Read the model definition and answer for the solid it produces. Units are mm, in the model's axes. Coordinates: 2 decimals unless noted, no trailing zeros. Loops run counter-clockwise (first coordinate to the right, second up) from the corner with the lowest first, then second, coordinate; pieces in that order, holes last. Notation, with made-up numbers: M -32,18.5 L -12,18.5 A16 ccw -12,27.5 Z; hole C 35.25,65 d7. An arc over 180 degrees is marked long. Put each result on its own line as item: value.
from build123d import *

# Parameters (mm, degrees)
SKETCH_1_R           = 21
BOSS_EXTRUDE_1_DEPTH = 16.5


with BuildPart() as part:
    # Sketch 1 → Boss-Extrude 1 (new, symmetric)
    with BuildSketch(Plane(origin=(0, 0, 0), x_dir=(1, 0, 0), z_dir=(0, 1, 0))):
        Polygon((0, 36.950417228), (-32, 18.475208614), (-32, -18.475208614), (0, -36.950417228), (32, -18.475208614), (32, 18.475208614), align=None)
        with Locations(Location((0, 0, 0), (0, 0, 270))):
            Circle(SKETCH_1_R, mode=Mode.SUBTRACT)
    extrude(amount=BOSS_EXTRUDE_1_DEPTH, both=True)

    # Sketch 2 → Cut-Revolve 1 (revolve, cut)
    with BuildSketch(Plane(origin=(0, 0, 0), x_dir=(0, 0, -1), z_dir=(1, 0, 0))):
        with BuildLine():
            Line((-30.950417228, 16.5), (-36.950417228, 16.5))
            Line((-36.950417228, 16.5), (-36.950417228, 13.5))
            add(Edge.make_bspline(
                [(-36.950417228, 13.5), (-35.688982599, 15.62896823), (-33.371774895, 16.5), (-30.950417228, 16.5)],
                knots=[0, 0, 0, 0, 1, 1, 1, 1], degree=3))
        make_face()
        with BuildLine():
            Line((-36.950417228, -16.5), (-36.950417228, -13.5))
            add(Edge.make_bspline(
                [(-36.950417228, -13.5), (-35.688982599, -15.62896823), (-33.371774895, -16.5), (-30.950417228, -16.5)],
                knots=[0, 0, 0, 0, 1, 1, 1, 1], degree=3))
            Line((-30.950417228, -16.5), (-36.950417228, -16.5))
        make_face()
    revolve(axis=Axis((0, 20.720193417, 0), (0, -1, 0)), mode=Mode.SUBTRACT)


solid = part.part
1) Given pin 1 Ø1.5 at (x, y) = (22, -13) entering from +Z; pin 2 Ø12 at (x, y) = (15, 1) entering from -Z, each flat-ended and moving along its own axis, determine where each tip first touches the part or whether it passes through.
Answer list:
pin 1: stops at z = 24.68
pin 2: stops at z = -31.75
2) Determine the mould class of faces 1 (the flat face through (-15.78, 0.23, -27.84)), 2 (the flat face through (6.4, 16.5, 20.2)), 3 (the cylindrical face through (6.31, -0.23, 20.03)) for opening direction X: released by +X, released by -X, zero draft, split by the parting line, or undercut.
Answer list:
face 1: released by -X
face 2: zero draft
face 3: undercut
3) Find section A-A, the plane y = -3. Write down the section's boundary in (x, z).
Answer list:
outline: M -32,-18.48 L 0,-36.95 L 32,-18.48 L 32,18.48 L 0,36.95 L -32,18.48 Z; hole C 0,0 d42
4) Straight lines are drawn through the part: line 1 (X direction, y = 6, z = 0); line 2 (X direction, y = -4, z = -10); line 3 (Z direction, x = -6, y = -14). For each, find the intervals that lie inside material, in ascending order. Write a range as [from, to].
Answer list:
line 1: x = [-32, -21], [21, 32]
line 2: x = [-32, -18.47], [18.47, 32]
line 3: z = [-33.49, -20.12], [20.12, 33.49]
